CAD build for the part. Positions are in the model's coordinates, mm. A direction names the side the tool comes from. Coordinates: 2 decimals unless noted, no trailing zeros. Loops run counter-clockwise (first coordinate to the right, second up) from the corner with the lowest first, then second, coordinate; pieces in that order, holes last. Notation, with made-up numbers: (31.5, -26) -> (88.5, -26) arc R15 ccw to (88.5, -6) -> close; hole circle Ø6 at (33, 47). An arc over 180 degrees is marked (long way). Write each question's results on one line, items separated by ' | '.
```python
from build123d import *

# Parameters (mm, degrees)
BRACKET_PLATE_PROFILE_R     = 4
BRACKET_PLATE_DEPTH         = 25
FORK_SLOT_SKETCH_W          = 80.7543585
FORK_SLOT_SKETCH_H          = 21.257894267
FORK_SLOT_DEPTH             = 108.407683018
PIVOT_BOSS_SKETCH_R         = 11
PIVOT_BOSS_22_DEPTH         = 30
PIVOT_BORE_SKETCH_R         = 7.5
PIVOT_BORE_15_DEPTH         = 131.686611628
FORK_NOTCH_SKETCH_W         = 22
FORK_NOTCH_SKETCH_H         = 19.498267172
FORK_NOTCH_22X10_DEPTH      = 109.680312712
FORK_PIN_HOLE_SKETCH_R      = 2
FORK_PIN_HOLE_DEPTH         = 30
CLAMP_HOLE_SKETCH_R         = 3
CLAMP_HOLE_DEPTH            = 30
CLAMP_POCKET_SKETCH_W       = 7.221877003
CLAMP_POCKET_SKETCH_H       = 6
CLAMP_POCKET_7_5_DEEP_DEPTH = 7.5
HOLE_12_SKETCH_R            = 6
HOLE_12_DEPTH               = 10


with BuildPart() as part:
    # Bracket Plate Profile → Bracket Plate (new body)
    with BuildSketch(Plane.XY):
        with BuildLine():
            Line((0, 0), (-72.873763146, 0))
            ThreePointArc((-72.873763146, 0), (-82.303926322, 3.335008681), (-87.540799358, 11.857063669))
            Line((-87.540799358, 11.857063669), (-97.364307589, 57.700102084))
            ThreePointArc((-97.364307589, 57.700102084), (-95.154146662, 65.077436074), (-87.743012223, 67.171464359))
            Line((-87.743012223, 67.171464359), (-41.201123946, 56.431028603))
            ThreePointArc((-41.201123946, 56.431028603), (-36.739368705, 53.616310244), (-35, 48.635899037))
            Line((-35, 48.635899037), (-35, 30))
            Line((-35, 30), (0, 30))
            Line((0, 30), (0, 21))
            Line((0, 21), (-22, 21))
            Line((-22, 21), (-22, 9))
            Line((-22, 9), (0, 9))
            Line((0, 9), (0, 0))
        make_face()
        with Locations((-89.541888277, 59.376334794)):
            Circle(BRACKET_PLATE_PROFILE_R, mode=Mode.SUBTRACT)
        with Locations((-43, 48.635899037)):
            Circle(BRACKET_PLATE_PROFILE_R, mode=Mode.SUBTRACT)
    extrude(amount=BRACKET_PLATE_DEPTH)

    # Fork Slot Sketch → Fork Slot (cut, through all)
    with BuildSketch(Plane(origin=(0, 30, 0), x_dir=(1, 0, 0), z_dir=(0, 1, 0))):
        with Locations((-75.37717925, -4.371052867)):
            Rectangle(FORK_SLOT_SKETCH_W, FORK_SLOT_SKETCH_H)
    extrude(amount=FORK_SLOT_DEPTH, mode=Mode.SUBTRACT)

    # Pivot Boss Sketch → Pivot Boss Ø22 (add)
    with BuildSketch(Plane(origin=(0, 0, 0), x_dir=(-1, 0, 0), z_dir=(0, 0, -1))):
        with Locations((72.873763146, 15)):
            Circle(PIVOT_BOSS_SKETCH_R)
    extrude(amount=PIVOT_BOSS_22_DEPTH)

    # Pivot Bore Sketch → Pivot Bore Ø15 (cut, through all)
    with BuildSketch(Plane(origin=(0, 0, -30), x_dir=(-1, 0, 0), z_dir=(0, 0, -1))):
        with Locations((72.873763146, 15)):
            Circle(PIVOT_BORE_SKETCH_R)
    extrude(amount=-PIVOT_BORE_15_DEPTH, mode=Mode.SUBTRACT)

    # Fork Notch Sketch → Fork Notch 22x10 (cut, through all)
    with BuildSketch(Plane(origin=(0, 30, 0), x_dir=(1, 0, 0), z_dir=(0, 1, 0))):
        with Locations((-11, -0.250866414)):
            Rectangle(FORK_NOTCH_SKETCH_W, FORK_NOTCH_SKETCH_H)
    extrude(amount=-FORK_NOTCH_22X10_DEPTH, mode=Mode.SUBTRACT)

    # Fork Pin Hole Sketch → Fork Pin Hole (cut)
    with BuildSketch(Plane(origin=(0, 30, 0), x_dir=(1, 0, 0), z_dir=(0, 1, 0))):
        with Locations(Location((-7, -17.5, 0), (0, 0, 180))):
            Circle(FORK_PIN_HOLE_SKETCH_R)
    extrude(amount=-FORK_PIN_HOLE_DEPTH, mode=Mode.SUBTRACT)

    # Clamp Hole Sketch → Clamp Hole (cut)
    with BuildSketch(Plane.XY.offset(25)):
        with Locations((-27, 15)):
            Circle(CLAMP_HOLE_SKETCH_R)
    extrude(amount=-CLAMP_HOLE_DEPTH, mode=Mode.SUBTRACT)

    # Clamp Pocket Sketch → Clamp Pocket 7.5 Deep (cut)
    with BuildSketch(Plane.XY.offset(25)):
        with Locations((-23.389061498, 15)):
            Rectangle(CLAMP_POCKET_SKETCH_W, CLAMP_POCKET_SKETCH_H)
    extrude(amount=-CLAMP_POCKET_7_5_DEEP_DEPTH, mode=Mode.SUBTRACT)

    # Hole Ø12 Sketch → Hole Ø12 (cut)
    with BuildSketch(Plane(origin=(0, 0, 0), x_dir=(-1, 0, 0), z_dir=(0, 0, -1))):
        with Locations((27, 15)):
            Circle(HOLE_12_SKETCH_R)
    extrude(amount=-HOLE_12_DEPTH, mode=Mode.SUBTRACT)


solid = part.part
```
Q1. Cut at C-C on y = 15. Write the cut outline in (x, z).
Results are:
outline: (-88.21, 0) -> (-83.87, 0) -> (-83.87, -30) -> (-80.37, -30) -> (-80.37, 25) -> (-88.21, 25) -> close; (-65.37, -30) -> (-61.87, -30) -> (-61.87, 0) -> (-33, 0) -> (-33, 10) -> (-30, 10) -> (-30, 25) -> (-65.37, 25) -> close; (-24, 10) -> (-22, 10) -> (-22, 17.5) -> (-24, 17.5) -> close
Q2. Cut at D-D on x = -43.5. Write the cut outline in (y, z), and give its area (3 significant figures).
Results are:
outline: (0, 0) -> (30, 0) -> (30, 15) -> (44.67, 15) -> (44.67, 25) -> (0, 25) -> close; (52.6, 15) -> (56.96, 15) -> (56.96, 25) -> (52.6, 25) -> close | area: 940 mm^2
Q3. Cut at B-B on z = 11.5. Write the cut outline in (x, y), and give its area (3 significant figures).
Results are:
outline: (-91.43, 30) -> (-87.54, 11.86) arc R15 ccw to (-72.87, 0) -> (0, 0) -> (0, 9) -> (-22, 9) -> (-22, 21) -> (0, 21) -> (0, 30) -> close; hole circle Ø15 at (-72.87, 15); hole circle Ø6 at (-27, 15) | area: 2,150 mm^2
Q4. Cut at A-A on x = -7. Write the cut outline in (y, z).
Results are:
outline: (0, 10) -> (9, 10) -> (9, 15.5) -> (0, 15.5) -> close; (0, 19.5) -> (9, 19.5) -> (9, 25) -> (0, 25) -> close; (21, 10) -> (30, 10) -> (30, 15.5) -> (21, 15.5) -> close; (21, 19.5) -> (30, 19.5) -> (30, 25) -> (21, 25) -> close
Q5. Pull direction X, two halves, no side cores. Call faces 5 (the cylindrical face through (-85.85, 57.84, 19.93)), 6 (the cylindrical face through (-64.14, 8.31, -14.79)), 7 (the flat face through (-23, 15, 17.5)): +X half, -X half, draft (parallel to the pull), parting line (faces both ways), or undercut.
Results are:
face 5: undercut | face 6: parting line | face 7: draft
Q6. Which spindle directions (+Z, -Z, +X, -X, +Y, -Y) get a long thin tool onto all of the face, cutting with end or side? Do faces 1 (the flat face through (-35, 39, 20)), 2 (the flat face through (-30, 14, 10)), 3 (the flat face through (-25, 18, 21)), 4 (the flat face through (-11, 5, 10)). Say none if no direction does.
Results are:
face 1: +Z, -Z, +X, +Y | face 2: -Z | face 3: +Z, +X | face 4: -Z, +X, +Y, -Y
Q7. Wall check: L1, parallel to Y at x = -27, z = 15; L2, parallel to Y at x = -4.5, z = 16.5; L3, parallel to Y at x = -50.5, z = 2. Give the ranges that are in metal, low to high. Write a range as from..to.
Results are:
L1: 0..12, 18..30 | L2: 0..9, 21..30 | L3: 0..30
Q8. Drop flat-ended pins along their axis: pin 1 (11 mm diameter, centred on x = -27, y = 15, fed in from -Z); pin 2 (4 mm diameter, centred on x = -47.5, y = 51.5, fed in from -Z); pin 3 (16.5 mm diameter, centred on x = -6.5, z = 21, fed in from +Y); pin 4 (8 mm diameter, centred on x = -29.5, y = 53.5, fed in from -Z). Give the stop position or say it passes through.
Results are:
pin 1: z = 10 | pin 2: z = 15 | pin 3: y = 30 | pin 4: through
